```python
from build123d import *

# Parameters (mm, degrees)
EXTRUDE1_DEPTH    = 900
SKETCH2_OUTSIDE_W = 2163.11
SKETCH2_OUTSIDE_H = 463.11
EXTRUDE5_DEPTH    = 100


with BuildPart() as part:
    # Sketch1 → Extrude1 (new, symmetric)
    with BuildSketch(Plane(origin=(0, 0, 0), x_dir=(0, 0, -1), z_dir=(1, 0, 0))):
        with BuildLine():
            Line((-44, 47.3), (-44, -32))
            ThreePointArc((-44, -32), (-40.485281374, -40.485281374), (-32, -44))
            Line((-32, -44), (47.3, -44))
            ThreePointArc((47.3, -44), (49.209188309, -44.790811691), (50, -46.7))
            Line((50, -46.7), (50, -50))
            Line((50, -50), (-50, -50))
            Line((-50, -50), (-50, 50))
            Line((-50, 50), (-46.7, 50))
            ThreePointArc((-46.7, 50), (-44.790811691, 49.209188309), (-44, 47.3))
        make_face()
    extrude(amount=EXTRUDE1_DEPTH, both=True)

    # Sketch2 outside → Extrude5 (cut)
    with BuildSketch(Plane.XY.offset(50)):
        Rectangle(SKETCH2_OUTSIDE_W, SKETCH2_OUTSIDE_H)
        Polygon((-138.272358385, 50), (-900, 50), (-535.395927853, -330.516583835), align=None, mode=Mode.SUBTRACT)
    extrude(amount=-EXTRUDE5_DEPTH, mode=Mode.SUBTRACT)


solid = part.part
```
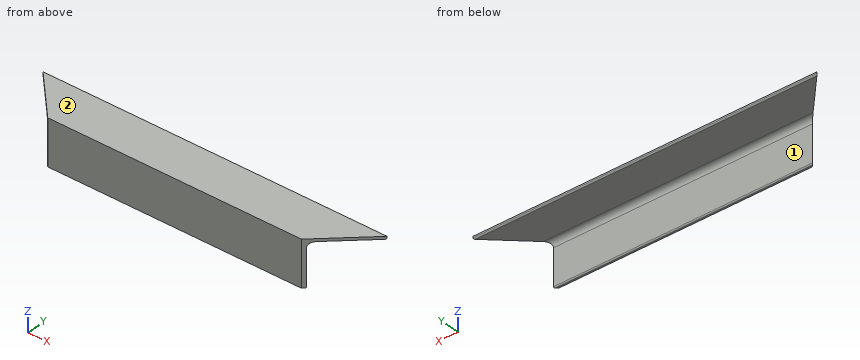
Build history of the part. All positions in model axes, mm. Face numbers are marked on the shaded views. A direction names the side the tool comes from. Give positions to 0.01 mm unless a question says otherwise; leave off trailing zeros. Loops run counter-clockwise (first coordinate to the right, second up) from the corner with the lowest first, then second, coordinate; pieces in that order, holes last. Notation, with made-up numbers: (70.5, 33) - (92.5, 33) arc R6 ccw to (92.5, 44) - close; hole circle Ø7 at (68, -5). An arc over 180 degrees is marked (long way). Use a Markdown table: item, result.
(1) Band-saw the part on D-D (x = -850). Give the cut face in (y, z).
Taken from the geometry:
| item | result |
|---|---|
| outline | (-2.18, 44) - (47.3, 44) arc R2.7 ccw to (50, 46.7) - (50, 50) - (-2.18, 50) - close |
(2) Band-saw the part on C-C (y = -11). Give the cut face in (x, z).
Taken from the geometry:
| item | result |
|---|---|
| outline | (-841.55, 44) - (-201.93, 44) - (-201.93, 50) - (-841.55, 50) - close |
(3) Band-saw the part on B-B (z = -41). Give the cut face in (x, y).
Taken from the geometry:
| item | result |
|---|---|
| outline | (-809.93, -44) - (-804.18, -50) - (-242.64, -50) - (-236.37, -44) - close |
(4) Wall check: line 1 along Z through (x, y) = (-241.5, 37); line 2 along Y through (x, z) = (-391.5, -8); line 3 along Y through (x, z) = (-687, 37). Give the ranges that are in metal, low to high.
Taken from the geometry:
| item | result |
|---|---|
| line 1 | 44 to 50 |
| line 2 | -50 to -44 |
| line 3 | -50 to -42.91 |
(5) Which spindle directions (+Z, -Z, +X, -X, +Y, -Y) get a long thin tool onto all of the face, cutting with end or side? Do the marked faces 1 and 2. Say none if no direction does.
Taken from the geometry:
| item | result |
|---|---|
| face 1 | -Z, +X, -X, +Y |
| face 2 | +Z, +X, -X, +Y, -Y |
(6) Band-saw the part on A-A (x = -658). Give the cut face in (y, z), and give its area (3 significant figures).
Taken from the geometry:
| item | result |
|---|---|
| outline | (-50, -50) - (-46.7, -50) arc R2.7 ccw to (-44, -47.3) - (-44, 32) arc R12 cw to (-32, 44) - (47.3, 44) arc R2.7 ccw to (50, 46.7) - (50, 50) - (-50, 50) - close |
| area | 1,190 mm2 |
(7) Drop flat-ended pins along their axis: pin 1 Ø24 at (x, z) = (-533, -24.5) entering from +Y; pin 2 Ø8 at (x, y) = (-667.5, -33) entering from -Z; pin 3 Ø6 at (x, y) = (-707.5, -10.5) entering from -Z. Give the stop position or say it passes through.
Taken from the geometry:
| item | result |
|---|---|
| pin 1 | y = -44 |
| pin 2 | z = 42.91 |
| pin 3 | z = 44 |
